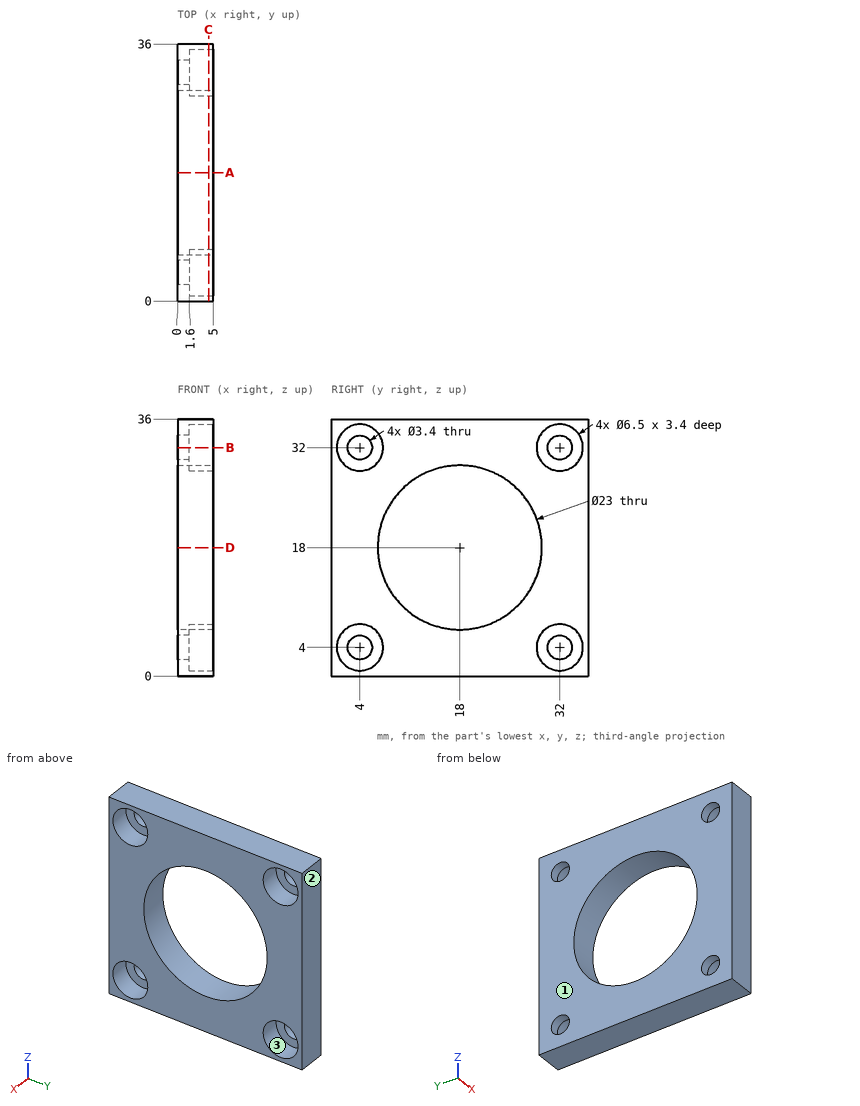
Study the drawing (mm; zero at the part's minimum x, y, z) and answer. Coordinates: 2 decimals unless noted, no trailing zeros. Order: outer loops, then holes, each group sorted by start corner. A loop starts at its lowest first (then second) coordinate and runs counter-clockwise, first axis right, second up. Notation, with made-up numbers: M 53,42 L 106,42 A24 ccw 106,71 Z; hole C -17.75,40.5 d11. An arc over 180 degrees is marked long. Answer as a JSON object with one key per item and string values. Group by question number.
1. Section A-A on y = 18 is taken. Write down the section's boundary in (x, z).
2. Determine the mould class of the marked faces 1, 2 and 3 for opening direction Y: released by +Y, released by -Y, zero draft, split by the parting line, or undercut.
3. Section C-C on x = 4.35 is taken. Write down the section's boundary in (y, z).
4. Straight lines are drawn through the part: line 1 (Y direction, x = 1.05, z = 32); line 2 (Y direction, x = 3.55, z = 4); line 3 (X direction, y = 2, z = 4.5). For each, find the intervals that lie inside material, in ascending order.
5. Section B-B on z = 32 is taken. Write down the section's boundary in (x, y), then the cut area to 3 significant figures.
6. Flat-ended cylindrical pins translate along their axes: P1, Ø5, axis at y = 4, z = 32, coming from the +X side; P2, Ø2, axis at y = 4, z = 32, coming from the -X side (1 decimal). Find the tip coordinate at first contact, or state that the pin passes through.
Values follow:
{
 "1": {"outline": "M 0,0 L 5,0 L 5,6.5 L 0,6.5 Z; M 0,29.5 L 5,29.5 L 5,36 L 0,36 Z"},
 "2": {"face 1": "zero draft", "face 2": "released by +Y", "face 3": "undercut"},
 "3": {"outline": "M 0,0 L 36,0 L 36,36 L 0,36 Z; hole C 4,4 d6.5; hole C 4,32 d6.5; hole C 18,18 d23; hole C 32,4 d6.5; hole C 32,32 d6.5"},
 "4": {"line 1": "0 to 2.3, 5.7 to 30.3, 33.7 to 36", "line 2": "0 to 0.75, 7.25 to 28.75, 35.25 to 36", "line 3": "0 to 1.6"},
 "5": {"outline": "M 0,0 L 5,0 L 5,0.75 L 1.6,0.75 L 1.6,2.3 L 0,2.3 Z; M 0,5.7 L 1.6,5.7 L 1.6,7.25 L 5,7.25 L 5,28.75 L 1.6,28.75 L 1.6,30.3 L 0,30.3 Z; M 0,33.7 L 1.6,33.7 L 1.6,35.25 L 5,35.25 L 5,36 L 0,36 Z", "area": "125 mm2"},
 "6": {"P1": "x = 1.6", "P2": "through"}
}
